The listing builds one solid part. Answer for the finished solid, in the listing's coordinates (mm). A direction names the side the tool comes from. Round coordinates to 2 decimals unless told otherwise and drop trailing zeros. Order: outer loops, then holes, each group sorted by start corner. A loop starts at its lowest first (then second) coordinate and runs counter-clockwise, first axis right, second up. Notation, with made-up numbers: M 62,-10 L 81,-10 A11 cw 81,-1 Z; hole C 81.5,58.25 d9. An arc over 180 degrees is marked long. Put each result on its own line as item: value. Start each with the question number.
1. The part is cut by section D-D (y = 15.5). Give the vertices of the cut face in (x, z).
2. Each of these flat-tipped pins is pushed along its axis until it touches: pin 1 Ø1 at (x, z) = (25.5, -23.5) entering from +Y; pin 2 Ø18 at (x, z) = (60, -30) entering from -Y; pin 3 Ø3 at (x, y) = (-1, -25.5) entering from -Z; pin 4 Ø2 at (y, z) = (-97, -11.5) entering from -X. Where does it stop, or does it pass through?
3. Which of the six approach directions +Z, -Z, +X, -X, +Y, -Y give full straight-line access (tool end or side, diameter ignored) to faces 1 (the face through (39.923, -60.56, -20.765)), 2 (the face through (15, 10, -53)), 3 (the face through (24.84, -6.9, -12.92)), 4 (the face through (-15, 10, -53))?
4. The part is cut by section B-B (z = 0). Count the separate pieces of the cut face and the enclosed holes in it, then the cut area to 3 significant figures.
5. The part is cut by section A-A (x = 60). Give the vertices of the cut face in (y, z).
6. Consider line 1 (X direction, y = -6.5, z = -30); line 2 (X direction, y = -8, z = 0); line 3 (Z direction, x = 60, y = -11.75). Determine where each line is inside the solid, lowest interval first.
7. The mould has two halves that part along X. Classify faces 5 (the face through (-90, -10, -1)), 6 (the face through (-69.76, -10.14, -2.17)), 7 (the face through (90, -10, 1)): +X half, -X half, draft (parallel to the pull), parting line (faces both ways), or undercut.
8. The part is cut by section C-C (z = -31.5). Give the vertices of the cut face in (x, y).
from build123d import *

# Parameters (mm, degrees)
FLANGE_START               = -20
FLANGE_PLATE_SKETCH_R      = 15
FLANGE_PLATE_SKETCH_R_2    = 10
FLANGE_PLATE_SKETCH_R_3    = 45
FLANGE_PLATE_120X180_DEPTH = 20
EYELET_LUG_SKETCH_R        = 10
EYELET_LUG_DEPTH           = 15


with BuildPart() as part:
    # Bushing Profile Sketch → Bushing Body (revolve)
    with BuildSketch(Plane.XY, mode=Mode.PRIVATE) as bushing_body_sk:
        Polygon((45, 0), (45, -100), (40, -100), (40, -110), (45, -110), (45, -135), (20, -135), (20, -14), (28, -14), (28, 0), align=None)
    revolve(bushing_body_sk.sketch.rotate(Axis((0, -88.636319954, 0), (0, 1, 0)), 90), axis=Axis((0, -88.636319954, 0), (0, 1, 0)))

    # Flange Plate Sketch → Flange Plate 120x180 (add)
    with BuildSketch(Plane(origin=(0, 0, 0), x_dir=(1, 0, 0), z_dir=(0, 1, 0)).offset(FLANGE_START)):
        with BuildLine():
            Line((-75, -60), (75, -60))
            ThreePointArc((75, -60), (85.606601718, -55.606601718), (90, -45))
            Line((90, -45), (90, 45))
            ThreePointArc((90, 45), (85.606601718, 55.606601718), (75, 60))
            Line((75, 60), (-75, 60))
            ThreePointArc((-75, 60), (-85.606601718, 55.606601718), (-90, 45))
            Line((-90, 45), (-90, -45))
            ThreePointArc((-90, -45), (-85.606601718, -55.606601718), (-75, -60))
        make_face()
        with Locations(Location((-60, -30, 0), (0, 0, 270))):
            Circle(FLANGE_PLATE_SKETCH_R, mode=Mode.SUBTRACT)
        with Locations(Location((-60, 0, 0), (0, 0, 270))):
            Circle(FLANGE_PLATE_SKETCH_R_2, mode=Mode.SUBTRACT)
        with Locations(Location((-60, 30, 0), (0, 0, 270))):
            Circle(FLANGE_PLATE_SKETCH_R, mode=Mode.SUBTRACT)
        with Locations(Location((60, -30, 0), (0, 0, 90))):
            Circle(FLANGE_PLATE_SKETCH_R, mode=Mode.SUBTRACT)
        with Locations(Location((60, 0, 0), (0, 0, 90))):
            Circle(FLANGE_PLATE_SKETCH_R_2, mode=Mode.SUBTRACT)
        with Locations(Location((60, 30, 0), (0, 0, 90))):
            Circle(FLANGE_PLATE_SKETCH_R, mode=Mode.SUBTRACT)
        with Locations(Location((0, 0, 0), (0, 0, 90))):
            Circle(FLANGE_PLATE_SKETCH_R_3, mode=Mode.SUBTRACT)
    extrude(amount=FLANGE_PLATE_120X180_DEPTH)

    # Eyelet Lug Sketch → Eyelet Lug (add)
    with BuildSketch(Plane(origin=(0, 0, -60), x_dir=(-1, 0, 0), z_dir=(0, 0, -1))):
        with BuildLine():
            Line((-15, 20), (-15, 0))
            Line((-15, 0), (15, 0))
            Line((15, 0), (15, 20))
            ThreePointArc((15, 20), (0, 35), (-15, 20))
        make_face()
        with Locations((0, 20)):
            Circle(EYELET_LUG_SKETCH_R, mode=Mode.SUBTRACT)
    extrude(amount=-EYELET_LUG_DEPTH)


solid = part.part
Resolved:
1. outline: M -15,-60 L -8.93,-60 L -8.93,-45 L -15,-45 Z; M 8.93,-60 L 15,-60 L 15,-45 L 8.93,-45 Z
2. pin 1: y = 0
2. pin 2: through
2. pin 3: z = -45
2. pin 4: x = -43.76
3. face 1: -Y
3. face 2: +Z, -Z, +X, +Y
3. face 3: +Y
3. face 4: +Z, -Z, -X, +Y
4. separate pieces: 4
4. enclosed holes: 0
4. area: 7,430 mm2
5. outline: M -20,-60 L 0,-60 L 0,-45 L -20,-45 Z; M -20,-15 L 0,-15 L 0,-10 L -20,-10 Z; M -20,10 L 0,10 L 0,15 L -20,15 Z; M -20,45 L 0,45 L 0,60 L -20,60 Z
6. line 1: -90 to -75, -45 to 45, 75 to 90
6. line 2: -90 to -70, -50 to -28, 28 to 50, 70 to 90
6. line 3: -60 to -45, -15 to -10, 10 to 15, 45 to 60
7. face 5: -X half
7. face 6: undercut
7. face 7: +X half
8. outline: M -90,-20 L -74.92,-20 L -74.92,0 L -90,0 Z; M -45.08,-20 L -32.14,-20 L -32.14,-100 L -24.65,-100 L -24.65,-110 L -32.14,-110 L -32.14,-135 L 32.14,-135 L 32.14,-110 L 24.65,-110 L 24.65,-100 L 32.14,-100 L 32.14,-20 L 45.08,-20 L 45.08,0 L -45.08,0 Z; M 74.92,-20 L 90,-20 L 90,0 L 74.92,0 Z
